```python
from build123d import *

# Parameters (mm, degrees)
SKETCH_2_R          = 2
CUT_EXTRUDE_1_DEPTH = 10
CHAMFER_1_SIZE      = 1


with BuildPart() as part:
    # 草图1 → 旋转1 (revolve)
    with BuildSketch(Plane.XY, mode=Mode.PRIVATE) as revolve_1_sk:
        Polygon((0, 29.25), (0, -29.25), (10, -29.25), (10, -25.75), (9, -25.75), (9, 1.25), (7.5, 1.25), (7.5, 29.25), align=None)
    revolve(revolve_1_sk.sketch.rotate(Axis((0, 29.25, 0), (0, -1, 0)), 180), axis=Axis((0, 29.25, 0), (0, -1, 0)))

    # 草图2 → 切除-拉伸1 (cut, symmetric)
    with BuildSketch(Plane(origin=(0, 0, 0), x_dir=(0, 0, -1), z_dir=(1, 0, 0))):
        with Locations((0, 23.75)):
            Circle(SKETCH_2_R)
    extrude(amount=CUT_EXTRUDE_1_DEPTH, both=True, mode=Mode.SUBTRACT)

    # 倒角1
    chamfer_1_edges = [part.edges().sort_by_distance(p)[0] for p in [
        (10, -29.25, 0),
        (7.5, 29.25, 0),
    ]]
    chamfer(chamfer_1_edges, length=CHAMFER_1_SIZE)


solid = part.part
```
Geometry check sheet. Reference: the model listing, model coordinates, mm. A direction names the side the tool comes from. Round coordinates to 2 decimals unless told otherwise and drop trailing zeros. Order: outer loops, then holes, each group sorted by start corner. A loop starts at its lowest first (then second) coordinate and runs counter-clockwise, first axis right, second up. Notation, with made-up numbers: (-16.75, -34.75) - (-7.75, -34.75) arc R15 cw to (-7.75, -29.75) - close; hole circle Ø5 at (-36, 20.25). An arc over 180 degrees is marked (long way). Use a Markdown table: item, result. Add a question column.
1) Mould release check, pull along Z, two halves, no side actions. Record for faces 1 (the cylindrical face through (6.633, -12.061, -6.083)), 2 (the cylindrical face through (0.105, 21.976, -0.923)), 3 (the flat face through (9, -25.75, -2)): released by +Z, released by -Z, zero draft, split by the parting line, or undercut.
2) Gauge pin test, flat ends, axial feed: P1, Ø4, axis at y = -16.5, z = -1, coming from the -X side; P2, Ø5, axis at y = -18.5, z = 6, coming from the -X side; P3, Ø5, axis at y = -5, z = -6.5, coming from the +X side. Record the tip position at first contact, or that the pin passes through.
3) Set-up check for faces 4 (the flat face through (0, 29.25, 0)), 5 (the flat face through (2, 1.25, -7.4)): record each of +Z, -Z, +X, -X, +Y, -Y from which the full face is reachable in a straight line by a thin tool's end or side.
4) Section check C-C (y = 4). Record the cut outline in (x, z), then the cut area to 3 significant figures.
5) Thickness scan on line 1 along Y through (x, z) = (1, 0); line 2 along Z through (x, y) = (-0.25, 23.75); line 3 along Z through (x, y) = (4.25, 23.75). Record the ranges inside material, lowest first.
6) Section check A-A (z = 0). Record the cut outline in (x, y).
7) Section check D-D (y = 23.75). Record the cut outline in (x, z), then the cut area to 3 significant figures.
8) Section check B-B (x = 0). Record the cut outline in (y, z).
Established:
| question | item | result |
|---|---|---|
| 1 | face 1 | split by the parting line |
| 1 | face 2 | undercut |
| 1 | face 3 | zero draft |
| 2 | P1 | x = -9 |
| 2 | P2 | x = -8.29 |
| 2 | P3 | x = 8.06 |
| 3 | face 4 | +Z, -Z, +X, -X, +Y |
| 3 | face 5 | +Y |
| 4 | outline | circle Ø15 at (0, 0) |
| 4 | area | 177 mm2 |
| 5 | line 1 | -29.25 to 21.75, 25.75 to 29.25 |
| 5 | line 2 | -7.5 to -2, 2 to 7.5 |
| 5 | line 3 | -6.18 to -2, 2 to 6.18 |
| 6 | outline | (-10, -28.25) - (-9, -29.25) - (9, -29.25) - (10, -28.25) - (10, -25.75) - (9, -25.75) - (9, 1.25) - (7.5, 1.25) - (7.5, 21.75) - (-7.5, 21.75) - (-7.5, 1.25) - (-9, 1.25) - (-9, -25.75) - (-10, -25.75) - close; (-7.5, 25.75) - (7.5, 25.75) - (7.5, 28.25) - (6.5, 29.25) - (-6.5, 29.25) - (-7.5, 28.25) - close |
| 7 | outline | (-7.23, -2) arc R7.5 ccw to (7.23, -2) - close; (-7.23, 2) - (7.23, 2) arc R7.5 ccw to start |
| 7 | area | 117 mm2 |
| 8 | outline | (-29.25, -9) - (-28.25, -10) - (-25.75, -10) - (-25.75, -9) - (1.25, -9) - (1.25, -7.5) - (28.25, -7.5) - (29.25, -6.5) - (29.25, 6.5) - (28.25, 7.5) - (1.25, 7.5) - (1.25, 9) - (-25.75, 9) - (-25.75, 10) - (-28.25, 10) - (-29.25, 9) - close; hole circle Ø4 at (23.75, 0) |
